CAD build for the part. Positions are in the model's coordinates, mm. Coordinates: 2 decimals unless noted, no trailing zeros. Loops run counter-clockwise (first coordinate to the right, second up) from the corner with the lowest first, then second, coordinate; pieces in that order, holes last. Notation, with made-up numbers: (-22.5, -12) -> (6.5, -12) arc R30 ccw to (6.5, 13) -> close; hole circle Ø4 at (41.5, 48). An arc over 180 degrees is marked (long way). Write item = value, one per line. Start each with the question number.
(1) Band-saw the part on C-C (z = -9.5). Write the cut outline in (x, y), and give its area (3 significant figures).
(2) Flat gauge pins, fed straight in: P1, Ø1.5, axis at x = 17.5, y = 29, coming from the +Z side; P2, Ø5, axis at x = 6.5, z = -0.5, coming from the +Y side; P3, Ø1, axis at x = -9, z = 18, coming from the +Y side; P4, Ø6, axis at x = 0, y = 0, coming from the -Z side. Where does each tip first touch, or does it go through?
(3) Band-saw the part on D-D (z = 12). Write the cut outline in (x, y).
(4) Pull direction Y, two halves, no side cores. Call faces 1 (the face through (17, 19, 0)), 2 (the face through (-0.54, -2.44, 6.9)), 3 (the face through (23.846, 7.509, 12.325)): +Y half, -Y half, draft (parallel to the pull), parting line (faces both ways), or undercut.
(5) Band-saw the part on A-A (x = 0). Write the cut outline in (y, z), and give its area (3 significant figures).
(6) Band-saw the part on B-B (y = 0). Write the cut outline in (x, z), and give its area (3 significant figures).
(7) Drill centre lines: line 1 (Y direction, x = 0, z = 21); line 2 (Y direction, x = 0, z = -2); line 3 (Z direction, x = -7.5, y = 37). Where is each one in solid material? Low to high. Write a range as from..to.
```python
from build123d import *

# Parameters (mm, degrees)
SKETCH1_R           = 25
BOSS_EXTRUDE1_DEPTH = 35
CHAMFER1_SIZE       = 10
CHAMFER1_SIZE2      = 6
SKETCH2_R           = 40
BOSS_EXTRUDE2_DEPTH = 22
SKETCH3_W           = 90
SKETCH3_H           = 30
CUT_EXTRUDE1_DEPTH  = 30
CHAMFER2_SIZE       = 2
M6_TAPPED_HOLE1_D   = 5


with BuildPart() as part:
    # Sketch1 → Boss-Extrude1 (new body)
    with BuildSketch(Plane.XY):
        Circle(SKETCH1_R)
    extrude(amount=BOSS_EXTRUDE1_DEPTH)

    # Chamfer1
    chamfer1_edges = [part.edges().sort_by_distance(p)[0] for p in [
        (-25, 0, 35),
    ]]
    chamfer1_side = [part.faces().sort_by_distance(p)[0] for p in [
        (-25, 0, 17.5),
    ]]
    chamfer(chamfer1_edges, length=CHAMFER1_SIZE, length2=CHAMFER1_SIZE2, reference=chamfer1_side[0])

    # Sketch2 → Boss-Extrude2 (add)
    with BuildSketch(Plane(origin=(0, 0, 0), x_dir=(-1, 0, 0), z_dir=(0, 0, -1))):
        Circle(SKETCH2_R)
    extrude(amount=BOSS_EXTRUDE2_DEPTH)

    # Sketch3 → Cut-Extrude1 (cut, symmetric)
    with BuildSketch(Plane(origin=(0, 0, 0), x_dir=(0, 0, -1), z_dir=(1, 0, 0))):
        with Locations((-23, -47)):
            Rectangle(SKETCH3_W, SKETCH3_H)
    extrude(amount=CUT_EXTRUDE1_DEPTH, both=True, mode=Mode.SUBTRACT)

    # Chamfer2
    chamfer2_edges = [part.edges().sort_by_distance(p)[0] for p in [
        (0, 40, 0),
    ]]
    chamfer(chamfer2_edges, length=CHAMFER2_SIZE)

    # M6 Tapped Hole1 (through all)
    with Locations(Plane(origin=(0, 0, -22), x_dir=(-1, 0, 0), z_dir=(0, 0, -1))):
        with Locations((0, 0)):
            Hole(M6_TAPPED_HOLE1_D / 2)


solid = part.part
```
Findings below:
q1.outline = (-24, -32) -> (24, -32) arc R40 ccw (long way) to start; hole circle Ø5 at (0, 0)
q1.area = 4,750 mm²
q2.P1 = 0
q2.P2 = 39.75
q2.P3 = 23.51
q2.P4 = -22
q3.outline = circle Ø50 at (0, 0); hole circle Ø5 at (0, 0)
q4.face_1 = draft
q4.face_2 = undercut
q4.face_3 = parting line
q5.outline = (-32, -22) -> (-2.5, -22) -> (-2.5, 35) -> (-19, 35) -> (-25, 25) -> (-25, 0) -> (-32, 0) -> close; (2.5, -22) -> (40, -22) -> (40, -2) -> (38, 0) -> (25, 0) -> (25, 25) -> (19, 35) -> (2.5, 35) -> close
q5.area = 2,990 mm²
q6.outline = (-40, -22) -> (-2.5, -22) -> (-2.5, 35) -> (-19, 35) -> (-25, 25) -> (-25, 0) -> (-38, 0) -> (-40, -2) -> close; (2.5, -22) -> (40, -22) -> (40, -2) -> (38, 0) -> (25, 0) -> (25, 25) -> (19, 35) -> (2.5, 35) -> close
q6.area = 3,160 mm²
q7.line_1 = -25..-2.5, 2.5..25
q7.line_2 = -32..-2.5, 2.5..40
q7.line_3 = -22..0
